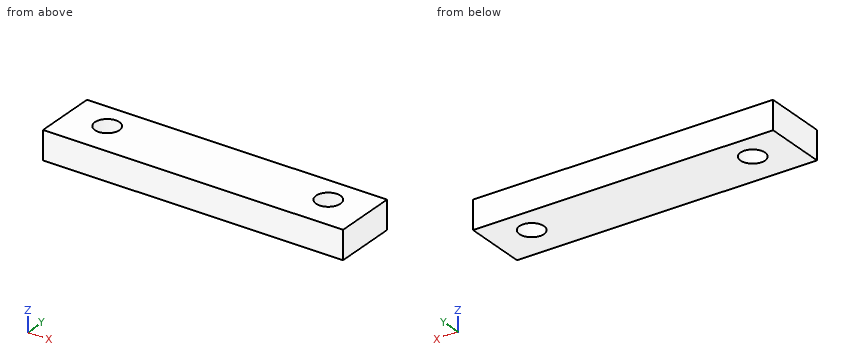
```python
from build123d import *

# Parameters (mm, degrees)
SKETCH1_W                = 380
SKETCH1_H                = 80
BOSS_EXTRUDE1_DEPTH      = 18
F_1_3_8_6_TAPPED_HOLE1_D = 30.95752


with BuildPart() as part:
    # Sketch1 → Boss-Extrude1 (new, symmetric)
    with BuildSketch(Plane.XY):
        Rectangle(SKETCH1_W, SKETCH1_H)
    extrude(amount=BOSS_EXTRUDE1_DEPTH, both=True)

    # 1-3/8-6 Tapped Hole1 (through all)
    with Locations(Plane.XY.offset(18)):
        with Locations((-140, 5), (140, 5)):
            Hole(F_1_3_8_6_TAPPED_HOLE1_D / 2)


solid = part.part
```
CAD build for the part. Positions are in the model's coordinates, mm. Round coordinates to 2 decimals unless told otherwise and drop trailing zeros. Write each loop counter-clockwise with the first axis right and the second up, starting at its lowest first coordinate (ties: lowest second). Pieces come first, ordered by that corner, then holes. Notation, with made-up numbers: (-18.75, 47) - (31.25, 47) arc R22 cw to (31.25, 72) - close; hole circle Ø5 at (22, 86). An arc over 180 degrees is marked (long way). Write item = value, one per line. Start each with the question number.
Q1. Band-saw the part on A-A (y = 5). Give the cut face in (x, z).
Q2. Band-saw the part on C-C (z = -10.5). Give the cut face in (x, y).
Q3. Band-saw the part on B-B (x = -140). Give the cut face in (y, z).
Q4. Probe L1, parallel to Y at x = 140, z = 9; L2, parallel to X at y = -9, z = -0.5; L3, parallel to Y at x = 136, z = 6. List the from-to ranges inside material, lowest first. Write a range as from..to.
Q5. Drop a flat-ended pin along its axis: pin 1 (18.5 mm diameter, centred on x = 140, y = 5, fed in from -Z). Give the stop position or say it passes through.
Answers below:
q1.outline = (-190, -18) - (-155.48, -18) - (-155.48, 18) - (-190, 18) - close; (-124.52, -18) - (124.52, -18) - (124.52, 18) - (-124.52, 18) - close; (155.48, -18) - (190, -18) - (190, 18) - (155.48, 18) - close
q2.outline = (-190, -40) - (190, -40) - (190, 40) - (-190, 40) - close; hole circle Ø30.96 at (-140, 5); hole circle Ø30.96 at (140, 5)
q3.outline = (-40, -18) - (-10.48, -18) - (-10.48, 18) - (-40, 18) - close; (20.48, -18) - (40, -18) - (40, 18) - (20.48, 18) - close
q4.L1 = -40..-10.48, 20.48..40
q4.L2 = -190..-146.6, -133.4..133.4, 146.6..190
q4.L3 = -40..-9.95, 19.95..40
q5.pin_1 = through
